CAD build for the part. Positions are in the model's coordinates, mm. A direction names the side the tool comes from. Round coordinates to 2 decimals unless told otherwise and drop trailing zeros. Write each loop counter-clockwise with the first axis right and the second up, starting at its lowest first coordinate (ties: lowest second). Pieces come first, ordered by that corner, then holes. Notation, with made-up numbers: (35.25, 83.5) - (61.25, 83.5) arc R31 ccw to (61.25, 114.5) - close; hole circle Ø6 at (30, 29). An arc over 180 degrees is marked (long way). Put each result on its own line as item: value. Start each with the question number.
Item 1: Pin check, flat tips, straight feed: pin 1 Ø1 at (x, y) = (18.5, 5) entering from -Z; pin 2 Ø3 at (x, y) = (-2.5, 3.5) entering from +Z; pin 3 Ø7 at (x, z) = (-25, 0) entering from -Y. Stop position of each tip, or through.
Item 2: Mould opens along Z. For faces 1 (the cylindrical face through (1.32, 3.45, -29.97)), 2 (the flat face through (0.3, 5.5, 4.2)), 3 (the flat face through (0, 0, 0)) say: released by +Z, released by -Z, zero draft, split by the parting line, or undercut.
Item 3: Drill centre lines: line 1 (Y direction, x = -13, z = -26); line 2 (Z direction, x = -24, y = 5.5); line 3 (Y direction, x = -7, z = -10.5). Where is each one in solid material? Low to high. Write a range as from..to.
Item 4: Cut at C-C (y = 3.5). Give the cut face in (x, z).
Item 5: Cut at D-D (z = 25). Give the cut face in (x, y), and give its area (3 significant figures).
Item 6: 3-axis set-ups, long thin cutter, end or side, ignore diameter. For faces 4 (the cylindrical face through (22, 4, 0)), 5 (the cylindrical face through (-19.524, 6.24, -4.336)): which of +Z, -Z, +X, -X, +Y, -Y reach the whole face in a straight line?
Item 7: Cut at B-B (z = 0). Give the cut face in (x, y), and give its area (3 significant figures).
Item 8: Cut at A-A (x = 0). Give the cut face in (y, z), and give its area (3 significant figures).
```python
from build123d import *

# Parameters (mm, degrees)
SKETCH1_R           = 30
BOSS_EXTRUDE1_DEPTH = 7
SKETCH2_R           = 4
BOSS_EXTRUDE2_DEPTH = 13
CUT_EXTRUDE1_START  = -1.5
SKETCH3_R           = 20
SKETCH3_R_2         = 4
CUT_EXTRUDE1_DEPTH  = 1.5
HOLE1_D             = 6
HOLE1_CSINK_D       = 9
HOLE1_CSINK_ANGLE   = 90
FILLET1_R           = 1.5


with BuildPart() as part:
    # Sketch1 → Boss-Extrude1 (new body)
    with BuildSketch(Plane(origin=(0, 0, 0), x_dir=(1, 0, 0), z_dir=(0, 1, 0))):
        with Locations(Location((0, 0, 0), (0, 0, 270))):
            Circle(SKETCH1_R)
    extrude(amount=BOSS_EXTRUDE1_DEPTH)

    # Sketch2 → Boss-Extrude2 (add)
    with BuildSketch(Plane(origin=(0, 7, 0), x_dir=(1, 0, 0), z_dir=(0, 1, 0))):
        with Locations(Location((0, 0, 0), (0, 0, 90))):
            Circle(SKETCH2_R)
    extrude(amount=BOSS_EXTRUDE2_DEPTH)

    # Sketch3 → Cut-Extrude1 (cut)
    with BuildSketch(Plane(origin=(0, 7, 0), x_dir=(1, 0, 0), z_dir=(0, 1, 0)).offset(CUT_EXTRUDE1_START)):
        with Locations(Location((0, 0, 0), (0, 0, 270))):
            Circle(SKETCH3_R)
        with Locations(Location((0, 0, 0), (0, 0, 90))):
            Circle(SKETCH3_R_2, mode=Mode.SUBTRACT)
    extrude(amount=CUT_EXTRUDE1_DEPTH, mode=Mode.SUBTRACT)

    # Hole1 (through all)
    with Locations(Plane(origin=(0, 0, 0), x_dir=(-1, 0, 0), z_dir=(0, -1, 0))):
        with Locations((-25, 0), (0, 25), (25, 0), (0, -25)):
            CounterSinkHole(HOLE1_D / 2, HOLE1_CSINK_D / 2, counter_sink_angle=HOLE1_CSINK_ANGLE)

    # Fillet1
    fillet1_edges = [part.edges().sort_by_distance(p)[0] for p in [
        (0, 20, 4),
    ]]
    fillet(fillet1_edges, radius=FILLET1_R)


solid = part.part
```
Output values:
1. pin 1: z = -24
1. pin 2: z = 29.98
1. pin 3: y = 1
2. face 1: split by the parting line
2. face 2: undercut
2. face 3: zero draft
3. line 1: 0..7
3. line 2: -18..-2.83, 2.83..18
3. line 3: 0..5.5
4. outline: circle Ø60 at (0, 0); hole circle Ø6 at (-25, 0); hole circle Ø6 at (0, -25); hole circle Ø6 at (0, 25); hole circle Ø6 at (25, 0)
5. outline: (-16.58, 0) - (-4.5, 0) - (-3, 1.5) - (-3, 7) - (-16.58, 7) - close; (3, 1.5) - (4.5, 0) - (16.58, 0) - (16.58, 7) - (3, 7) - close
5. area: 188 mm2
6. face 4: +Y, -Y
6. face 5: +Y
7. outline: (-30, 0) - (-29.5, 0) - (-28, 1.5) - (-28, 7) - (-30, 7) - close; (-22, 1.5) - (-20.5, 0) - (20.5, 0) - (22, 1.5) - (22, 7) - (20, 7) - (20, 5.5) - (4, 5.5) - (4, 18.5) arc R1.5 ccw to (2.5, 20) - (-2.5, 20) arc R1.5 ccw to (-4, 18.5) - (-4, 5.5) - (-20, 5.5) - (-20, 7) - (-22, 7) - close; (28, 1.5) - (29.5, 0) - (30, 0) - (30, 7) - (28, 7) - close
7. area: 387 mm2
8. outline: (0, -30) - (7, -30) - (7, -28) - (1.5, -28) - (0, -29.5) - close; (0, -20.5) - (1.5, -22) - (7, -22) - (7, -20) - (5.5, -20) - (5.5, -4) - (18.5, -4) arc R1.5 ccw to (20, -2.5) - (20, 2.5) arc R1.5 ccw to (18.5, 4) - (5.5, 4) - (5.5, 20) - (7, 20) - (7, 22) - (1.5, 22) - (0, 20.5) - close; (0, 29.5) - (1.5, 28) - (7, 28) - (7, 30) - (0, 30) - close
8. area: 387 mm2
